Work out the finished part from the listing and answer in its coordinate system (mm). A direction names the side the tool comes from. Coordinates: 2 decimals unless noted, no trailing zeros. Write each loop counter-clockwise with the first axis right and the second up, starting at its lowest first coordinate (ties: lowest second). Pieces come first, ordered by that corner, then holes. Notation, with made-up numbers: M 18.25,-12 L 23.25,-12 A17 ccw 23.25,4 Z; hole C 3,80 d11. An arc over 180 degrees is marked long. Use CSV: the item, a comma, the result in double quotes.
from build123d import *

# Parameters (mm, degrees)
SKETCH_1_W          = 30
SKETCH_1_H          = 30
SKETCH_1_W_2        = 26
SKETCH_1_H_2        = 26
EXTRUDE_1_DEPTH     = 833.5
CUT_EXTRUDE_1_DEPTH = 35
SKETCH_4_R          = 5.75
CUT_EXTRUDE_2_DEPTH = 163


with BuildPart() as part:
    # 草图1 → 凸台-拉伸1 (new, symmetric)
    with BuildSketch(Plane.XY):
        Rectangle(SKETCH_1_W, SKETCH_1_H)
        Rectangle(SKETCH_1_W_2, SKETCH_1_H_2, mode=Mode.SUBTRACT)
    extrude(amount=EXTRUDE_1_DEPTH, both=True)

    # 草图3 → 切除-拉伸1 (cut, symmetric)
    with BuildSketch(Plane(origin=(0, 15, 0), x_dir=(1, 0, 0), z_dir=(0, 1, 0))):
        Polygon((15, -833.5), (15, -778.5), (-15, -753.327011065), (-15, -833.5), align=None)
    extrude(amount=CUT_EXTRUDE_1_DEPTH, both=True, mode=Mode.SUBTRACT)

    # 草图4 → 切除-拉伸2 (cut)
    with BuildSketch(Plane.XZ.offset(15)):
        with Locations((0, 745.413505532)):
            Circle(SKETCH_4_R)
        with Locations((0, 720.413505532)):
            Circle(SKETCH_4_R)
    extrude(amount=-CUT_EXTRUDE_2_DEPTH, mode=Mode.SUBTRACT)


solid = part.part
Item 1: For a pull along X with two mould halves and no side action, classify faces 3 (the face through (-15, 0, -29)), 4 (the face through (15, 0, -16)), 5 (the face through (-13, 0, -28)), 6 (the face through (-14, 0, -833.5)) as released by +X, released by -X, zero draft, split by the parting line, or undercut.
Answer:
face 3,"released by -X"
face 4,"released by +X"
face 5,"undercut"
face 6,"zero draft"
Item 2: The part is cut by section B-B (z = 108.5). Write down the section's boundary in (x, y).
Answer:
outline,"M -15,-15 L 15,-15 L 15,15 L -15,15 Z; hole M -13,-13 L 13,-13 L 13,13 L -13,13 Z"
Item 3: Consider probe 1 along Y at (x, z) = (-5, -341.5); probe 2 along Z at (x, y) = (0, 14.45). Determine where each line is inside the solid, lowest interval first.
Answer:
probe 1,"y = -15 to -13, 13 to 15"
probe 2,"z = -833.5 to 714.66, 726.16 to 739.66, 751.16 to 765.91"
Item 4: Given pin 1 (10 mm diameter, centred on x = -1, y = -12, fed in from +Z), flat-ended and moving along its own axis, determine where the tip first touches the part or whether it passes through.
Answer:
pin 1,"stops at z = 769.19"
Item 5: The part is cut by section C-C (x = 0). Write down the section's boundary in (y, z).
Answer:
outline,"M -15,-833.5 L -13,-833.5 L -13,714.66 L -15,714.66 Z; M -15,726.16 L -13,726.16 L -13,739.66 L -15,739.66 Z; M -15,751.16 L -13,751.16 L -13,765.91 L -15,765.91 Z; M 13,-833.5 L 15,-833.5 L 15,714.66 L 13,714.66 Z; M 13,726.16 L 15,726.16 L 15,739.66 L 13,739.66 Z; M 13,751.16 L 15,751.16 L 15,765.91 L 13,765.91 Z"
Item 6: The part is cut by section A-A (y = -8.5). Write down the section's boundary in (x, z).
Answer:
outline,"M -15,-833.5 L -13,-833.5 L -13,755.01 L -15,753.33 Z; M 13,-833.5 L 15,-833.5 L 15,778.5 L 13,776.82 Z"
Item 7: A tool of negligible diameter and unlimited length cuts with its end or side. For faces 1 (the face through (0, 15, -16)), 2 (the face through (13, 0, -17)), from which of +Z, -Z, +X, -X, +Y, -Y can it reach the whole face along a straight path? Write none if from no direction.
Answer:
face 1,"+Z, -Z, +X, -X, +Y"
face 2,"+Z, -Z"
